Work out the finished part from the listing and answer in its coordinate system (mm). A direction names the side the tool comes from. Coordinates: 2 decimals unless noted, no trailing zeros. Order: outer loops, then holes, each group sorted by start corner. A loop starts at its lowest first (then second) coordinate and runs counter-clockwise, first axis right, second up. Notation, with made-up numbers: (31.5, 42.5) - (53.5, 42.5) arc R16 ccw to (53.5, 67.5) - close; hole circle Ø7 at (46, 2). An arc over 180 degrees is marked (long way). Answer as a JSON object with one key per item and string values. Group by question number.
1) Section D-D (x = 36) is taken. Give the vertices of the cut face in (y, z), plus the area to 3 significant figures.
2) Each of these flat-tipped pins is pushed along its axis until it touches: P1, Ø3, axis at y = -13, z = 32.5, coming from the -X side; P2, Ø3, axis at y = 55.5, z = 14.5, coming from the -X side; P3, Ø8, axis at x = 1, z = -9, coming from the +Y side; P4, Ø9, axis at x = 0, y = -50, coming from the +Z side. Where does it stop, or does it pass through?
3) A tool of negligible diameter and unlimited length cuts with its end or side. For faces 4 (the face through (1, -20, -19)), 5 (the face through (0.66, 90.14, -14.985)), 6 (the face through (0, -38, 10)), 7 (the face through (0, 0, 0)), 8 (the face through (-17.235, -9.86, -41.569)), from which of +Z, -Z, +X, -X, +Y, -Y can it reach the whole face along a straight path? Write none if from no direction.
4) Section B-B (z = 0) is taken. Give the vertices of the cut face in (x, y), plus the area to 3 significant figures.
5) The mould has two halves that part along Z. Classify faces 1 (the face through (0, -38, -10)), 2 (the face through (-1.63, -57.32, -0.14)), 3 (the face through (1.32, 40.56, -29.97)): released by +Z, released by -Z, zero draft, split by the parting line, or undercut.
6) Find the intervals of material crossed by line 1 along Y through (x, z) = (12, 12.5); line 2 along X through (y, z) = (86.25, 0); line 3 along X through (y, z) = (63, 0), in increasing order.
7) Section C-C (y = -50) is taken. Give the vertices of the cut face in (x, z), plus the area to 3 significant figures.
from build123d import *

# Parameters (mm, degrees)
SKETCH_1_R          = 40
EXTRUDE_1_DEPTH     = 80
SKETCH_2_R          = 45
EXTRUDE_2_DEPTH     = 20
EXTRUDE_START       = 20
SKETCH_3_R          = 45
EXTRUDE_3_DEPTH     = 20
CUT_EXTRUDE_START   = -20
SKETCH_4_R          = 30
CUT_EXTRUDE_2_DEPTH = 80
SKETCH_5_R          = 15
CUT_EXTRUDE_3_DEPTH = 40
SKETCH_6_R          = 7.5
EXTRUDE_4_DEPTH     = 10
FILLET_1_R          = 2


with BuildPart() as part:
    # 草图1 → 凸台-拉伸1 (new body)
    with BuildSketch(Plane(origin=(0, 0, 0), x_dir=(1, 0, 0), z_dir=(0, 1, 0))):
        with Locations(Location((0, 0, 0), (0, 0, 270))):
            Circle(SKETCH_1_R)
    extrude(amount=EXTRUDE_1_DEPTH)

    # 草图2 → 凸台-拉伸2 (add)
    with BuildSketch(Plane.XZ):
        with Locations(Location((0, 0, 0), (0, 0, 270))):
            Circle(SKETCH_2_R)
    extrude(amount=EXTRUDE_2_DEPTH)

    # 草图3 → 凸台-拉伸3 (add)
    with BuildSketch(Plane(origin=(0, 80, 0), x_dir=(1, 0, 0), z_dir=(0, 1, 0)).offset(EXTRUDE_START)):
        with Locations(Location((0, 0, 0), (0, 0, 90))):
            Circle(SKETCH_3_R)
    extrude(amount=-EXTRUDE_3_DEPTH)

    # 草图4 → 切除-拉伸2 (cut)
    with BuildSketch(Plane(origin=(0, 100, 0), x_dir=(1, 0, 0), z_dir=(0, 1, 0)).offset(CUT_EXTRUDE_START)):
        with Locations(Location((0, 0, 0), (0, 0, 270))):
            Circle(SKETCH_4_R)
    extrude(amount=-CUT_EXTRUDE_2_DEPTH, mode=Mode.SUBTRACT)

    # 草图5 → 切除-拉伸3 (cut)
    with BuildSketch(Plane(origin=(0, 100, 0), x_dir=(1, 0, 0), z_dir=(0, 1, 0))):
        with Locations(Location((0, 0, 0), (0, 0, 270))):
            Circle(SKETCH_5_R)
    extrude(amount=-CUT_EXTRUDE_3_DEPTH, mode=Mode.SUBTRACT)

    # 草图6 → 凸台-拉伸4 (add, symmetric)
    with BuildSketch(Plane.XY):
        with BuildLine():
            Line((-14.014695363, -55.346804082), (-27.5, -20))
            Line((-27.5, -20), (27.5, -20))
            Line((27.5, -20), (14.014695363, -55.346804082))
            ThreePointArc((14.014695363, -55.346804082), (0, -65), (-14.014695363, -55.346804082))
        make_face()
        with Locations((0, -50)):
            Circle(SKETCH_6_R, mode=Mode.SUBTRACT)
    extrude(amount=EXTRUDE_4_DEPTH, both=True)

    # 圆角1
    fillet_1_edges = [part.edges().sort_by_distance(p)[0] for p in [
        (0, -20, 10),
        (0, -20, -10),
        (27.5, -20, 0),
        (-27.5, -20, 0),
    ]]
    fillet(fillet_1_edges, radius=FILLET_1_R)


solid = part.part
Report:
{
 "1": {"outline": "(-20, -27) - (0, -27) - (0, -17.44) - (80, -17.44) - (80, -27) - (100, -27) - (100, 27) - (80, 27) - (80, 17.44) - (0, 17.44) - (0, 27) - (-20, 27) - close", "area": "4,950 mm²"},
 "2": {"P1": "stops at x = -32.62", "P2": "stops at x = -37.83", "P3": "stops at y = 0", "P4": "passes through"},
 "3": {"face 4": "-Y", "face 5": "+Y", "face 6": "+Z, +X, -X, -Y", "face 7": "none", "face 8": "+Y, -Y"},
 "4": {"outline": "(-45, -20) - (-28.88, -20) arc R2 cw to (-27.01, -21.29) - (-14.01, -55.35) arc R15 ccw to (14.01, -55.35) - (27.01, -21.29) arc R2 cw to (28.88, -20) - (45, -20) - (45, 0) - (40, 0) - (40, 80) - (45, 80) - (45, 100) - (15, 100) - (15, 80) - (30, 80) - (30, 0) - (-30, 0) - (-30, 80) - (-15, 80) - (-15, 100) - (-45, 100) - (-45, 80) - (-40, 80) - (-40, 0) - (-45, 0) - close; hole circle Ø15 at (0, -50)", "area": "6,090 mm²"},
 "5": {"face 1": "released by -Z", "face 2": "zero draft", "face 3": "undercut"},
 "6": {"line 1": "y = -20 to 0, 80 to 100", "line 2": "x = -45 to -15, 15 to 45", "line 3": "x = -40 to -30, 30 to 40"},
 "7": {"outline": "(-16.05, -10) - (-7.5, -10) - (-7.5, 10) - (-16.05, 10) - close; (7.5, -10) - (16.05, -10) - (16.05, 10) - (7.5, 10) - close", "area": "342 mm²"}
}
